```python
from build123d import *

# Parameters (mm, degrees)
EXTRUDE_1_DEPTH     = 6
SKETCH_2_R          = 2.25
CUT_EXTRUDE_1_DEPTH = 12
FILLET_1_R          = 3
FILLET_2_R          = 5
FILLET_3_R          = 5
FILLET_4_R          = 0.2


with BuildPart() as part:
    # 草图1 → 凸台-拉伸1 (new, symmetric)
    with BuildSketch(Plane(origin=(0, 0, 0), x_dir=(0, 0, -1), z_dir=(1, 0, 0))):
        with BuildLine():
            Line((43.757393596, 17.659225719), (60, 17.659225719))
            Line((60, 17.659225719), (60, 19.659225719))
            Line((60, 19.659225719), (45.097063909, 19.659225719))
            ThreePointArc((45.097063909, 19.659225719), (0, 49.195836501), (-45.097063909, 19.659225719))
            Line((-45.097063909, 19.659225719), (-60, 19.659225719))
            Line((-60, 19.659225719), (-60, 17.659225719))
            Line((-60, 17.659225719), (-43.757393596, 17.659225719))
            ThreePointArc((-43.757393596, 17.659225719), (0, 47.186414859), (43.757393596, 17.659225719))
        make_face()
    extrude(amount=EXTRUDE_1_DEPTH, both=True)

    # 草图2 → 切除-拉伸1 (cut)
    with BuildSketch(Plane(origin=(0, 19.659225719, 0), x_dir=(1, 0, 0), z_dir=(0, 1, 0))):
        with Locations(Location((0, -52.5, 0), (0, 0, 270))):
            Circle(SKETCH_2_R)
        with Locations(Location((0, 52.5, 0), (0, 0, 270))):
            Circle(SKETCH_2_R)
    extrude(amount=-CUT_EXTRUDE_1_DEPTH, mode=Mode.SUBTRACT)

    # 圆角1
    fillet_1_edges = [part.edges().sort_by_distance(p)[0] for p in [
        (6, 18.659225719, -60),
        (6, 18.659225719, 60),
        (-6, 18.659225719, 60),
        (-6, 18.659225719, -60),
    ]]
    fillet(fillet_1_edges, radius=FILLET_1_R)

    # 圆角2
    fillet_2_edges = [part.edges().sort_by_distance(p)[0] for p in [
        (0, 19.659225719, 45.097063909),
        (0, 19.659225719, -45.097063909),
    ]]
    fillet(fillet_2_edges, radius=FILLET_2_R)

    # 圆角3
    fillet_3_edges = [part.edges().sort_by_distance(p)[0] for p in [
        (0, 17.659225719, 43.757393596),
        (0, 17.659225719, -43.757393596),
    ]]
    fillet(fillet_3_edges, radius=FILLET_3_R)

    # 圆角4
    fillet_4_edges = [part.edges().sort_by_distance(p)[0] for p in [
        (6, 19.659225719, -52.630433487),
        (0, 19.659225719, 60),
        (-5.121320344, 19.659225719, 59.121320344),
        (5.121320344, 19.659225719, 59.121320344),
        (-6, 19.659225719, -52.630433487),
        (0, 19.659225719, -60),
        (5.121320344, 19.659225719, -59.121320344),
        (-5.121320344, 19.659225719, -59.121320344),
        (-6, 49.195836501, 0),
        (6, 49.195836501, 0),
        (6, 19.659225719, 52.630433487),
        (-6, 19.659225719, 52.630433487),
        (-6, 20.394541943, -45.650795653),
        (6, 20.394541943, -45.650795653),
        (-6, 20.394541943, 45.650795653),
        (6, 20.394541943, 45.650795653),
    ]]
    fillet(fillet_4_edges, radius=FILLET_4_R)


solid = part.part
```
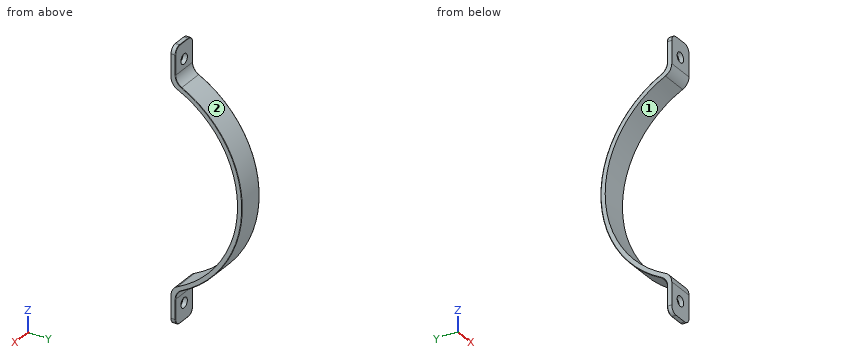
Read the model definition and answer for the solid it produces. Units are mm, in the model's axes. Face numbers are marked on the shaded views. Coordinates: 2 decimals unless noted, no trailing zeros. Write each loop counter-clockwise with the first axis right and the second up, starting at its lowest first coordinate (ties: lowest second). Pieces come first, ordered by that corner, then holes. Notation, with made-up numbers: (-9.75, -36.75) -> (40.25, -36.75) arc R23 cw to (40.25, -25.75) -> close; hole circle Ø2 at (8.5, 66.25). An arc over 180 degrees is marked (long way). Answer as a JSON object with one key per item and string values.
Q1. Determine the mould class of the marked faces 1 and 2 for opening direction Z: pulls with the +Z half, pulls with the -Z half, needs draft (parallel to the pull), parting line crosses it, or undercut.
The answers:
{"face 1": "undercut", "face 2": "parting line crosses it"}
Q2. The part is cut by section B-B on x = 0. Give the vertices of the cut face in (y, z), then the cut area to 3 significant figures.
The answers:
{"outline": "(17.66, -60) -> (19.46, -60) arc R0.2 ccw to (19.66, -59.8) -> (19.66, -54.75) -> (17.66, -54.75) -> close; (17.66, -50.25) -> (19.66, -50.25) -> (19.66, -48.26) arc R5 cw to (22.38, -43.81) arc R49.2 ccw to (22.38, 43.81) arc R5 cw to (19.66, 48.26) -> (19.66, 50.25) -> (17.66, 50.25) -> (17.66, 47.01) arc R5 ccw to (20.49, 42.51) arc R47.19 cw to (20.49, -42.51) arc R5 ccw to (17.66, -47.01) -> close; (17.66, 54.75) -> (19.66, 54.75) -> (19.66, 59.8) arc R0.2 ccw to (19.46, 60) -> (17.66, 60) -> close", "area": "271 mm2"}
Q3. Flat-ended cylindrical pins translate along their axes: pin 1 Ø4 at (y, z) = (24, -46) entering from -X; pin 2 Ø10 at (y, z) = (38, 23.5) entering from +X; pin 3 Ø5 at (x, z) = (-4, -29.5) entering from -Y; pin 4 Ø1 at (x, y) = (0, 40) entering from -Z. Find the tip coordinate at first contact, or state that the pin passes through.
The answers:
{"pin 1": "passes through", "pin 2": "stops at x = 6", "pin 3": "stops at y = 34.68", "pin 4": "stops at z = -29.33"}
Q4. Consider line 1 (X direction, y = 18.95, z = 52.5); line 2 (Y direction, x = -4, z = 52.5); line 3 (Y direction, x = 1, z = 0). Determine where each line is inside the solid, lowest interval first. Write a range as [from, to].
The answers:
{"line 1": "x = [-6, -2.25], [2.25, 6]", "line 2": "y = [17.66, 19.66]", "line 3": "y = [47.19, 49.2]"}
Q5. The part is cut by section A-A on z = 52.5. Give the vertices of the cut face in (x, y), then the cut area to 3 significant figures.
The answers:
{"outline": "(-6, 17.66) -> (-2.25, 17.66) -> (-2.25, 19.66) -> (-5.8, 19.66) arc R0.2 ccw to (-6, 19.46) -> close; (2.25, 17.66) -> (6, 17.66) -> (6, 19.46) arc R0.2 ccw to (5.8, 19.66) -> (2.25, 19.66) -> close", "area": "15.0 mm2"}
